Could you check a few things on this drawing? It's one solid part, dimensions in mm from its lowest x, y, z. A direction names the side the tool comes from. Round coordinates to 2 decimals unless told otherwise and drop trailing zeros. Loops run counter-clockwise (first coordinate to the right, second up) from the corner with the lowest first, then second, coordinate; pieces in that order, holes last. Notation, with made-up numbers: M 9,-2.5 L 49,-2.5 A23 ccw 49,27.5 Z; hole C 10,23.25 d1. An arc over 180 degrees is marked long. Answer as a JSON object with one key per item and string values.
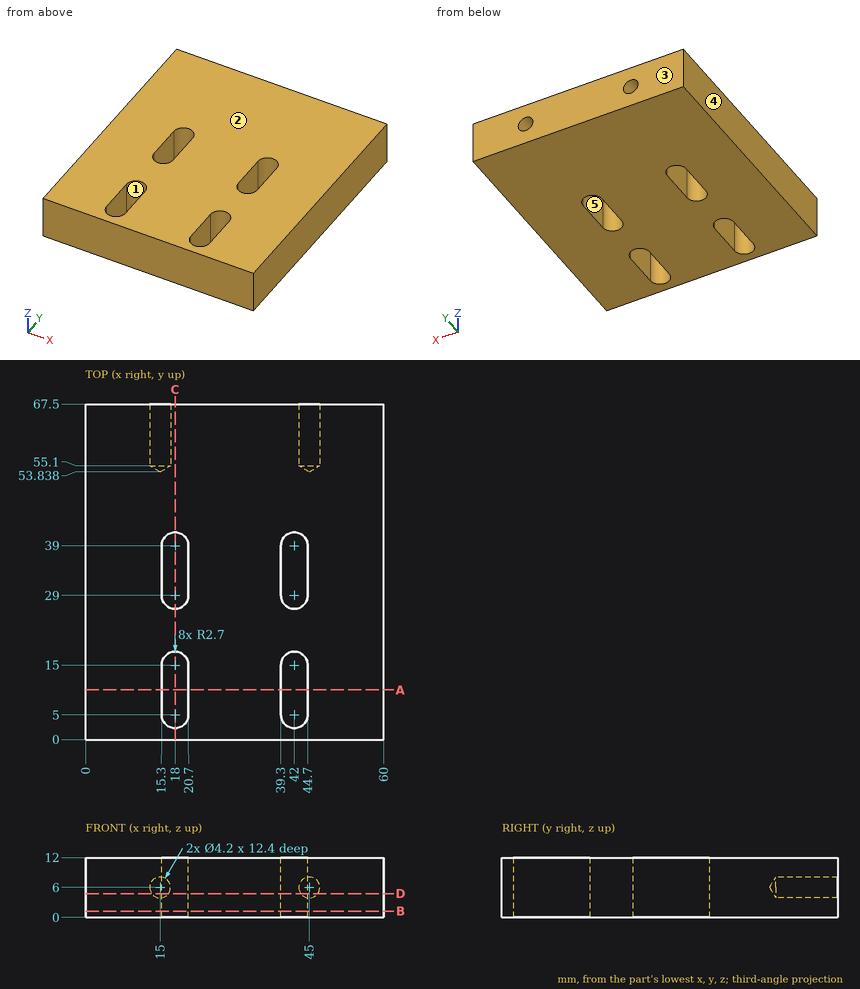
Item 1: I want a section at B-B, the plane z = 1.25. Please give me the cut outline in (x, y), then the cut area to 3 significant figures.
Resolved:
{"outline": "M 0,0 L 60,0 L 60,67.5 L 0,67.5 Z; hole M 15.3,5 A2.7 ccw 20.7,5 L 20.7,15 A2.7 ccw 15.3,15 Z; hole M 15.3,29 A2.7 ccw 20.7,29 L 20.7,39 A2.7 ccw 15.3,39 Z; hole M 39.3,5 A2.7 ccw 44.7,5 L 44.7,15 A2.7 ccw 39.3,15 Z; hole M 39.3,29 A2.7 ccw 44.7,29 L 44.7,39 A2.7 ccw 39.3,39 Z", "area": "3,740 mm²"}
Item 2: I want a section at D-D, the plane z = 4.75. State how many separate pieces and enclosed holes the cut face has, then the cut area to 3 significant figures.
Resolved:
{"separate pieces": "1", "enclosed holes": "4", "area": "3,660 mm²"}
Item 3: I want a section at C-C, the plane x = 18. Please give me the cut outline in (y, z), then the cut area to 3 significant figures.
Resolved:
{"outline": "M 0,0 L 2.3,0 L 2.3,12 L 0,12 Z; M 17.7,0 L 26.3,0 L 26.3,12 L 17.7,12 Z; M 41.7,0 L 67.5,0 L 67.5,12 L 41.7,12 Z", "area": "440 mm²"}
Item 4: I want a section at A-A, the plane y = 10. Please give me the cut outline in (x, z), then the cut area to 3 significant figures.
Resolved:
{"outline": "M 0,0 L 15.3,0 L 15.3,12 L 0,12 Z; M 20.7,0 L 39.3,0 L 39.3,12 L 20.7,12 Z; M 44.7,0 L 60,0 L 60,12 L 44.7,12 Z", "area": "590 mm²"}
Item 5: Please list where these lines run through material, in increasing order: probe 1 along X at (y, z) = (14, 10.5); probe 2 along Y at (x, z) = (42, 10); probe 3 along Z at (x, y) = (45, 60.75). Write a range as from..to.
Resolved:
{"probe 1": "0..15.3, 20.7..39.3, 44.7..60", "probe 2": "0..2.3, 17.7..26.3, 41.7..67.5", "probe 3": "0..3.9, 8.1..12"}
Item 6: If we mould it in two halves opening along Y, with no side actions, what happens to the marked faces 3, 4 and 5? For each: pulls with the +Y half, pulls with the -Y half, needs draft (parallel to the pull), parting line crosses it, or undercut.
Resolved:
{"face 3": "pulls with the +Y half", "face 4": "needs draft", "face 5": "undercut"}
Item 7: On a 3-axis mill with a long thin cutter (end or side, diameter ignored), from which of +Z, -Z, +X, -X, +Y, -Y can I reach the whole of each face in a straight line? I mean the marked faces 1 and 2. Say none if no direction works.
Resolved:
{"face 1": "+Z, -Z", "face 2": "+Z, +X, -X, +Y, -Y"}
